CAD build for the part. Positions are in the model's coordinates, mm. Face numbers are marked on the shaded views. A direction names the side the tool comes from. Give positions to 0.01 mm unless a question says otherwise; leave off trailing zeros. Write each loop counter-clockwise with the first axis right and the second up, starting at its lowest first coordinate (ties: lowest second). Pieces come first, ordered by that corner, then holes. Notation, with made-up numbers: (43.25, -28) - (52.25, -28) arc R16 cw to (52.25, -12) - close; hole circle Ø1 at (69, -15.75). An arc over 180 degrees is marked (long way). Answer as a JSON object with one key per item and string values.
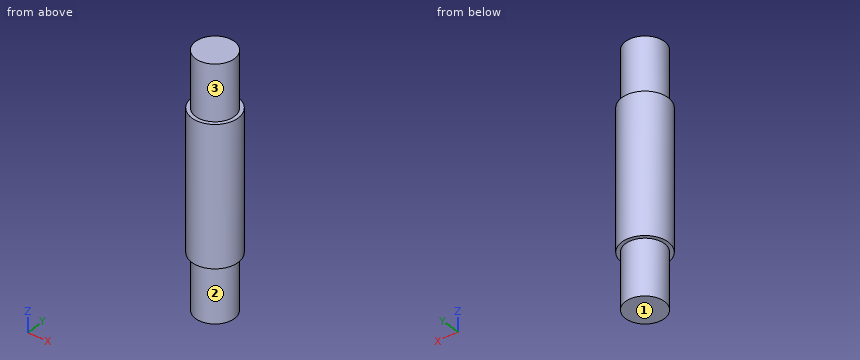
from build123d import *

# Parameters (mm, degrees)
SKETCH_1_R           = 25
BOSS_EXTRUDE_1_DEPTH = 75
SKETCH_2_R           = 21
BOSS_EXTRUDE_2_DEPTH = 60


with BuildPart() as part:
    # Sketch 1 → Boss-Extrude 1 (new, symmetric)
    with BuildSketch(Plane.XY):
        Circle(SKETCH_1_R)
    extrude(amount=BOSS_EXTRUDE_1_DEPTH, both=True)

    # Sketch 2 → Boss-Extrude 2 (add)
    with BuildSketch(Plane.XY.offset(75)):
        Circle(SKETCH_2_R)
    boss_extrude_2 = extrude(amount=BOSS_EXTRUDE_2_DEPTH)

    # Mirror 1: Boss-Extrude 2 across plane
    add(boss_extrude_2.mirror(Plane.XY))


solid = part.part
(1) Flat gauge pins, fed straight in: P1, Ø1, axis at y = -18.5, z = -95, coming from the +X side; P2, Ø4, axis at y = 7.5, z = -2.5, coming from the -X side; P3, Ø10, axis at x = 4, z = 39, coming from the +Y side. Where does each tip first touch, or does it go through?
Answer key:
{"P1": "stops at x = 10.82", "P2": "stops at x = -24.39", "P3": "stops at y = 25"}
(2) 3-axis set-ups, long thin cutter, end or side, ignore diameter. For the marked faces 1, 2 and 3: which of +Z, -Z, +X, -X, +Y, -Y reach the whole face in a straight line?
Answer key:
{"face 1": "-Z, +X, -X, +Y, -Y", "face 2": "-Z", "face 3": "+Z"}
(3) Saw through at D-D, the plane z = -54.5. Give the cut face in (x, y), and give its area (3 significant figures).
Answer key:
{"outline": "circle Ø50 at (0, 0)", "area": "1,960 mm²"}
(4) Saw through at C-C, the plane z = -99. Give the cut face in (x, y), and give its area (3 significant figures).
Answer key:
{"outline": "circle Ø42 at (0, 0)", "area": "1,390 mm²"}
(5) Saw through at A-A, the plane x = 0. Give the cut face in (y, z).
Answer key:
{"outline": "(-25, -75) - (-21, -75) - (-21, -135) - (21, -135) - (21, -75) - (25, -75) - (25, 75) - (21, 75) - (21, 135) - (-21, 135) - (-21, 75) - (-25, 75) - close"}
(6) Probe L1, parallel to Z at x = -12.5, y = 17; L2, parallel to X at y = -6, z = 106; L3, parallel to X at y = 6, z = 8. List the from-to ranges inside material, lowest first. Write a range as [from, to].
Answer key:
{"L1": "z = [-75, 75]", "L2": "x = [-20.12, 20.12]", "L3": "x = [-24.27, 24.27]"}
